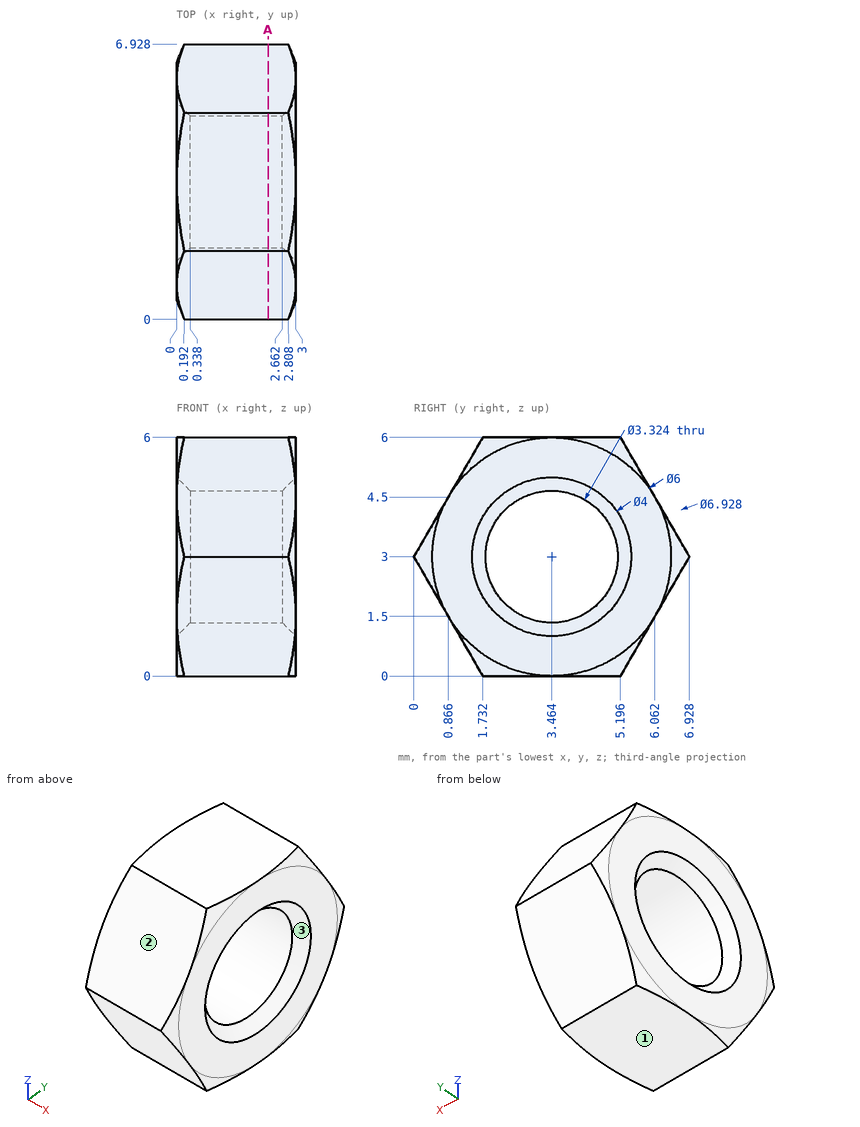
Could you check a few things on this drawing? It's one solid part, dimensions in mm from its lowest x, y, z. Give positions to 0.01 mm unless a question says otherwise; leave off trailing zeros. Loops run counter-clockwise (first coordinate to the right, second up) from the corner with the lowest first, then second, coordinate; pieces in that order, holes last. Notation, with made-up numbers: M -15,36 L 6,36 A14 cw 6,62 Z; hole C 54.25,-3.5 d9. An arc over 180 degrees is marked long. Return JSON: item names as keys, results as strings.
Item 1: I'm going to push a flat-ended pin straight in: pin 1 Ø1 at (x, z) = (2.5, 1) entering from -Y (1 decimal). Where does the tip first touch, or does it pass through?
A:
{"pin 1": "stops at y = 0.9"}
Item 2: Imagine slicing it at A-A on x = 2.3. List the corners of the cut face in (y, z) for me (1 decimal), then the cut area to 3 significant figures.
A:
{"outline": "M 0,3 L 1.7,0 L 5.2,0 L 6.9,3 L 5.2,6 L 1.7,6 Z; hole C 3.5,3 d3.3", "area": "22.5 mm^2"}
Item 3: Please list where these lines run through material, in increasing order: line 1 (Z direction, x = 2.55, y = 3.5); line 2 (Z direction, x = 1.75, y = 2.75); line 3 (Y direction, x = 0.7, z = 4.25) (1 decimal).
A:
{"line 1": "z = 0 to 1.34, 4.66 to 6", "line 2": "z = 0 to 1.5, 4.5 to 6", "line 3": "y = 0.7 to 2.4, 4.6 to 6.2"}
Item 4: Thinking about a two-plate mould opening in Y: for the marked faces 1, 2 and 3, which applies, released by +Y, released by -Y, zero draft, split by the parting line, or undercut?
A:
{"face 1": "zero draft", "face 2": "released by -Y", "face 3": "undercut"}
